Job drawing, mm, ordinate dimensions from the low corner. One solid piece. A direction names the side the tool comes from. Round coordinates to 2 decimals unless told otherwise and drop trailing zeros. Write each loop counter-clockwise with the first axis right and the second up, starting at its lowest first coordinate (ties: lowest second). Pieces come first, ordered by that corner, then holes. Notation, with made-up numbers: M -5.5,-32.5 L 45.5,-32.5 A21 cw 45.5,2.5 Z; hole C -35,68.5 d6. An arc over 180 degrees is marked long. One line per item, written item: value. Start each with the question number.
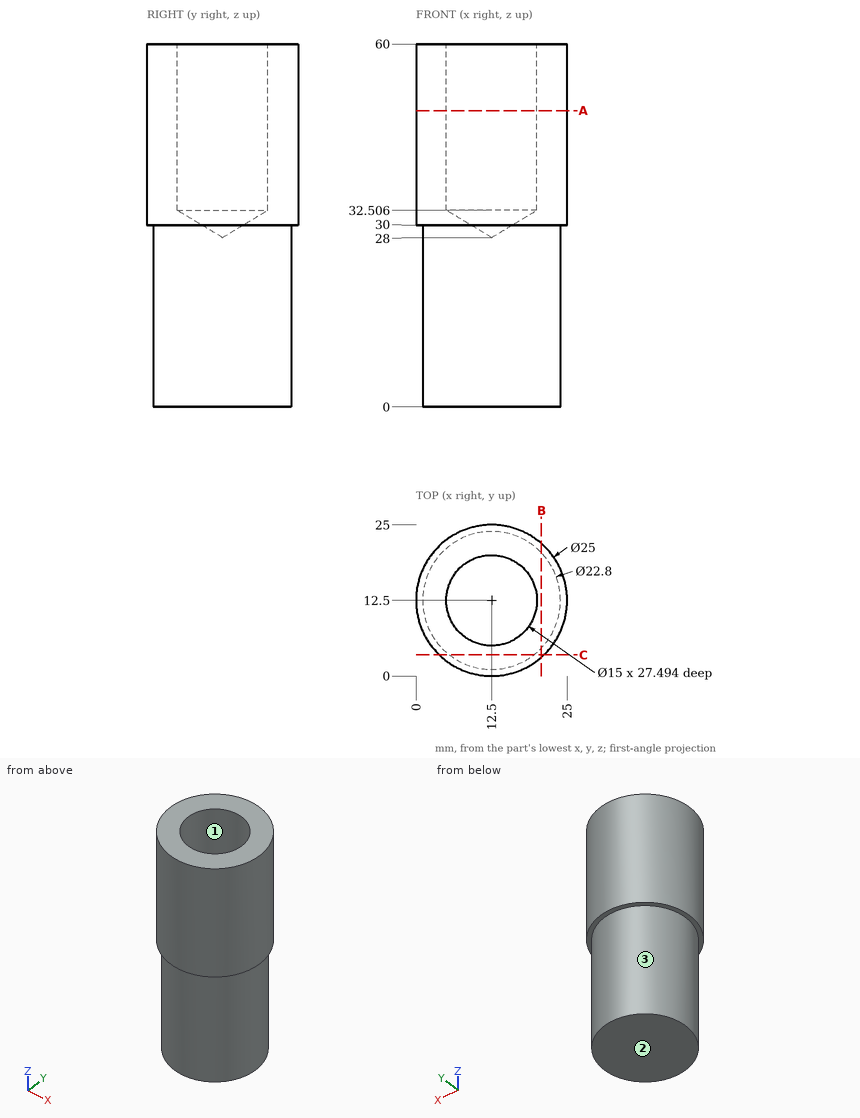
Item 1: Drop flat-ended pins along their axis: pin 1 (1.5 mm diameter, centred on y = 15.5, z = 43.5, fed in from -X); pin 2 (4 mm diameter, centred on y = 14, z = 18.5, fed in from +X); pin 3 (1.5 mm diameter, centred on x = 20, z = 28, fed in from -Y); pin 4 (12 mm diameter, centred on x = 8.5, z = 30, fed in from +Y). Give the stop position or say it passes through.
Item 2: Which spindle directions (+Z, -Z, +X, -X, +Y, -Y) get a long thin tool onto all of the face, cutting with end or side? Do the marked faces 1, 2 and 3. Say none if no direction does.
Item 3: Drill centre lines: line 1 (Y direction, x = 12.5, z = 50); line 2 (X direction, y = 17.75, z = 51) (1 decimal); line 3 (Z direction, x = 17.25, y = 2). Where is each one in solid material? Low to high.
Item 4: Cut at B-B, the plane x = 20.75. Write the cut outline in (y, z).
Item 5: Cut at C-C, the plane y = 3.5. Write the cut outline in (x, z) (1 decimal).
Item 6: Cut at A-A, the plane z = 49. Write the cut outline in (x, y).
Computed values:
1. pin 1: stops at x = 0.2
1. pin 2: stops at x = 23.9
1. pin 3: stops at y = 3.31
1. pin 4: stops at y = 25
2. face 1: +Z
2. face 2: -Z, +X, -X, +Y, -Y
2. face 3: -Z
3. line 1: y = 0 to 5, 20 to 25
3. line 2: x = 1.2 to 7.1, 17.9 to 23.8
3. line 3: z = 30 to 60
4. outline: M 3.11,30 L 4.63,30 L 4.63,0 L 20.37,0 L 20.37,30 L 21.89,30 L 21.89,60 L 3.11,60 Z
5. outline: M 3.8,30 L 5.5,30 L 5.5,0 L 19.5,0 L 19.5,30 L 21.2,30 L 21.2,60 L 3.8,60 Z
6. outline: C 12.5,12.5 d25; hole C 12.5,12.5 d15
